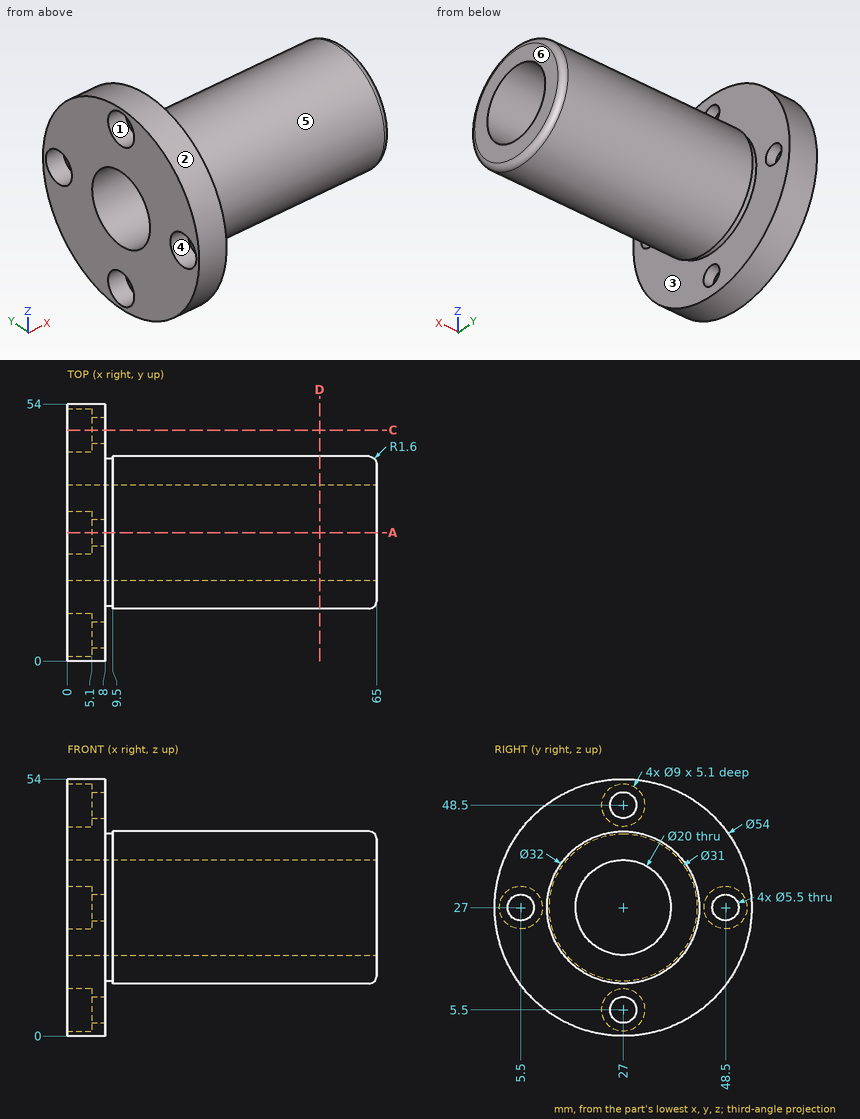
Drawing for the job (mm, zero at the part's lowest x, y, z). A direction names the side the tool comes from. Give positions to 0.01 mm unless a question says otherwise; leave off trailing zeros. Order: outer loops, then holes, each group sorted by start corner. A loop starts at its lowest first (then second) coordinate and runs counter-clockwise, first axis right, second up. Notation, with made-up numbers: M 6,-8 L 63,-8 A14 cw 63,15 Z; hole C 19,16.25 d5. An arc over 180 degrees is marked long. Use a Markdown table: item, result. Add a question column.
(1) Saw through at A-A, the plane y = 27. Give the number of separate pieces and of enclosed holes in the cut face, and give its area (3 significant figures).
(2) Probe line 1 along Y through (x, z) = (7.35, 27); line 2 along Y through (x, z) = (2.3, 27); line 3 along Y through (x, z) = (26, 27). List the from-to ranges inside material, lowest first. Write a range as [from, to].
(3) Drop flat-ended pins along their axis: P1, Ø11.5, axis at y = 5.5, z = 27, coming from the +X side; P2, Ø4.5, axis at y = 48, z = 25, coming from the -X side; P3, Ø5, axis at x = 38.5, z = 15, coming from the +Y side. Give the stop position or say it passes through.
(4) Saw through at C-C, the plane y = 48.5. Give the cut face in (x, z), and give its area (3 significant figures).
(5) Saw through at D-D, the plane x = 53. Give the cut face in (y, z), and give its area (3 significant figures).
(6) Mould opens along Y. For the marked faces 1, 2 and 3 say: +Y half, -Y half, draft (parallel to the pull), parting line (faces both ways), or undercut.
(7) 3-axis set-ups, long thin cutter, end or side, ignore diameter. For the marked faces 4, 5 and 6: which of +Z, -Z, +X, -X, +Y, -Y reach the whole face in a straight line?
Answer key:
| question | item | result |
|---|---|---|
| 1 | separate pieces | 4 |
| 1 | enclosed holes | 0 |
| 1 | area | 830 mm^2 |
| 2 | line 1 | [0, 2.75], [8.25, 17], [37, 45.75], [51.25, 54] |
| 2 | line 2 | [0, 1], [10, 17], [37, 44], [53, 54] |
| 2 | line 3 | [11, 17], [37, 43] |
| 3 | P1 | x = 64.26 |
| 3 | P2 | x = 5.1 |
| 3 | P3 | y = 39.87 |
| 4 | outline | M 0,10.67 L 8,10.67 L 8,24.25 L 5.1,24.25 L 5.1,22.5 L 0,22.5 Z; M 0,31.5 L 5.1,31.5 L 5.1,29.75 L 8,29.75 L 8,43.33 L 0,43.33 Z |
| 4 | area | 199 mm^2 |
| 5 | outline | C 27,27 d32; hole C 27,27 d20 |
| 5 | area | 490 mm^2 |
| 6 | face 1 | undercut |
| 6 | face 2 | parting line |
| 6 | face 3 | draft |
| 7 | face 4 | -X |
| 7 | face 5 | +X |
| 7 | face 6 | +Z, -Z, +X, +Y, -Y |
